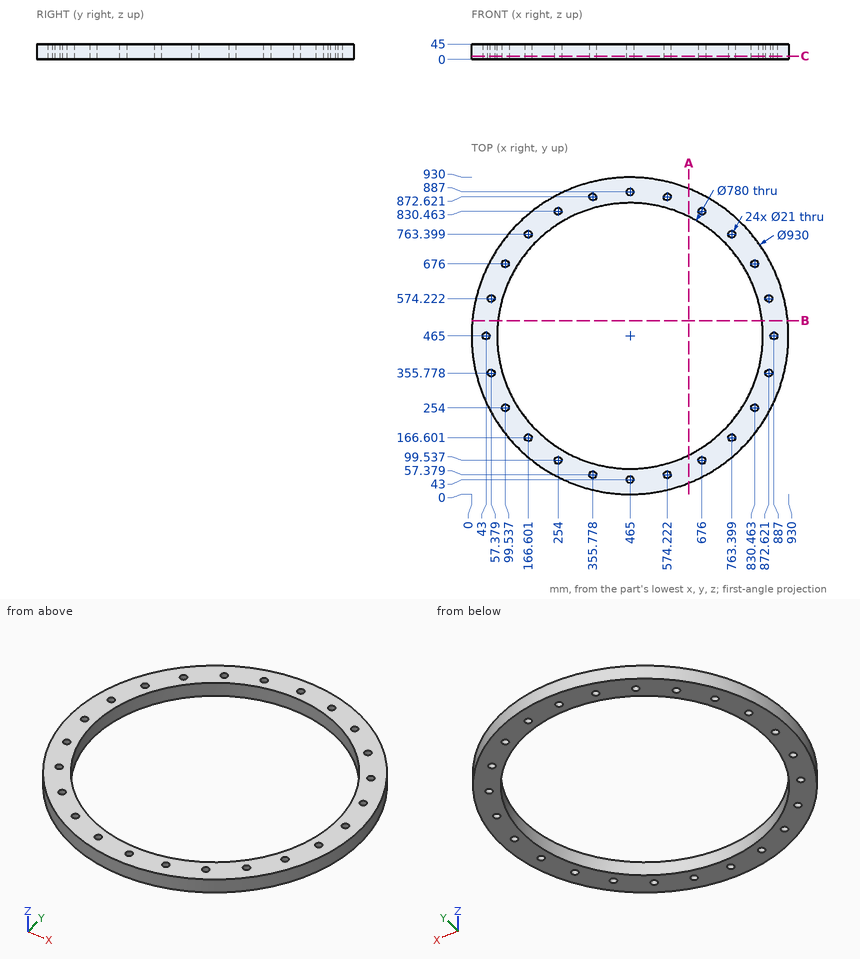
Could you check a few things on this drawing? It's one solid part, dimensions in mm from its lowest x, y, z. Coordinates: 2 decimals unless noted, no trailing zeros. Loops run counter-clockwise (first coordinate to the right, second up) from the corner with the lowest first, then second, coordinate; pieces in that order, holes last. Notation, with made-up numbers: (74, 68.5) - (104, 68.5) arc R14 ccw to (104, 87.5) - close; hole circle Ø11 at (-7.75, 66). An arc over 180 degrees is marked (long way). Answer as a JSON object with one key per item and string values. Group by question number.
Item 1: If we section it at B-B (y = 509.5): List the corners of the cut face in (x, z) for me.
Item 2: If we section it at A-A (x = 638): List the corners of the cut face in (y, z) for me, plus the area to 3 significant figures.
Item 3: If I drill on L1, parallel to X at y = 754.5, z = 22.5 (1 decimal); L2, parallel to Y at x = 566.5, z = 33 (1 decimal); L3, parallel to Y at x = 349, z = 31.5, over which ranges is the centre line in solid material (lowest first)? Write a range as from..to.
Item 4: For pin 1 (5 mm diameter, centred on y = 707, z = 40, fed in from -X); pin 2 (8 mm diameter, centred on y = 291.5, z = 8, fed in from +X); pin 3 (8 mm diameter, centred on x = 114, z = 37.5, fed in from +Y), each with a flat end and sliding along its axis, tell me the tip position at first contact or that it passes through.
Item 5: If we section it at C-C (z = 9.5): State how many separate pieces and enclosed holes the cut face has, plus the area to 3 significant figures.
Returned:
{
 "1": {"outline": "(2.13, 0) - (77.55, 0) - (77.55, 45) - (2.13, 45) - close; (852.45, 0) - (927.87, 0) - (927.87, 45) - (852.45, 45) - close"},
 "2": {"outline": "(33.38, 0) - (115.47, 0) - (115.47, 45) - (33.38, 45) - close; (814.53, 0) - (896.62, 0) - (896.62, 45) - (814.53, 45) - close", "area": "7,390 mm²"},
 "3": {"L1": "x = 101.1..161, 172.2..203.7, 726.3..757.8, 769..828.9", "L2": "y = 11.2..50.3, 64.5..88.4, 841.6..865.5, 879.7..918.8", "L3": "y = 14.7..49.36, 65.4..92.65, 837.35..864.6, 880.64..915.3"},
 "4": {"pin 1": "stops at x = 66.42", "pin 2": "stops at x = 898.01", "pin 3": "stops at y = 774.54"},
 "5": {"separate pieces": "1", "enclosed holes": "25", "area": "193,000 mm²"}
}
